Model file for the job. Use its own axes, mm. A direction names the side the tool comes from. Round coordinates to 2 decimals unless told otherwise and drop trailing zeros. Order: outer loops, then holes, each group sorted by start corner. A loop starts at its lowest first (then second) coordinate and runs counter-clockwise, first axis right, second up. Notation, with made-up numbers: (1, -3) - (46, -3) arc R23 cw to (46, 25) - close; hole circle Ø10 at (-14.75, -40). An arc over 180 degrees is marked (long way). Write item = value, one per line.
```python
from build123d import *

# Parameters (mm, degrees)
BOSS_EXTRUDE1_DEPTH   = 12.5
CHAMFER1_SIZE         = 2
HOLE1_D               = 9
CUT_EXTRUDE1_DEPTH    = 15
M4_TAPPED_HOLE1_D     = 3.3
SKETCH11_W            = 35
SKETCH11_H            = 25
CUT_EXTRUDE2_DEPTH    = 250.850455273
M8_TAPPED_HOLE2_D     = 6.8
M8_TAPPED_HOLE2_DEPTH = 19.75
M8_TAPPED_HOLE2_TIP   = 2.042926105


with BuildPart() as part:
    # Sketch1 → Boss-Extrude1 (new, symmetric)
    with BuildSketch(Plane(origin=(0, 0, 0), x_dir=(1, 0, 0), z_dir=(0, 1, 0))):
        Polygon((-75, 0), (75, 0), (75, 12), (40, 12), (40, 250), (-40, 250), (-40, 12), (-75, 12), align=None)
    extrude(amount=BOSS_EXTRUDE1_DEPTH, both=True)

    # Chamfer1
    chamfer1_edges = [part.edges().sort_by_distance(p)[0] for p in [
        (-75, 0, -12),
        (-40, 0, -250),
        (40, 0, -250),
        (75, 0, -12),
    ]]
    chamfer(chamfer1_edges, length=CHAMFER1_SIZE)

    # Hole1 (through all)
    with Locations(Plane.XY):
        with Locations((-60, 0), (60, 0)):
            Hole(HOLE1_D / 2)

    # Sketch4 → Cut-Extrude1 (cut)
    with BuildSketch(Plane(origin=(0, -12.5, 0), x_dir=(-1, 0, 0), z_dir=(0, -1, 0))):
        with BuildLine():
            Line((-13.5, 80), (-13.5, 250))
            ThreePointArc((-13.5, 250), (0, 263.5), (13.5, 250))
            Line((13.5, 250), (13.5, 80))
            ThreePointArc((13.5, 80), (0, 66.5), (-13.5, 80))
        make_face()
    extrude(amount=-CUT_EXTRUDE1_DEPTH, mode=Mode.SUBTRACT)

    # M4 Tapped Hole1 (through all)
    with Locations(Plane(origin=(0, 12.5, 0), x_dir=(1, 0, 0), z_dir=(0, 1, 0))):
        with Locations((-10, 235), (-10, 221), (10, 221), (10, 235)):
            Hole(M4_TAPPED_HOLE1_D / 2)

    # Sketch11 → Cut-Extrude2 (cut, through all)
    with BuildSketch(Plane(origin=(0, 0, -12), x_dir=(-1, 0, 0), z_dir=(0, 0, -1))):
        with Locations((-57.5, 0)):
            Rectangle(SKETCH11_W, SKETCH11_H)
        with Locations((57.5, 0)):
            Rectangle(SKETCH11_W, SKETCH11_H)
    extrude(amount=-CUT_EXTRUDE2_DEPTH, mode=Mode.SUBTRACT)

    # M8 Tapped Hole2
    with Locations(Plane.XY):
        with Locations((-25, 0), (25, 0)):
            Hole(M8_TAPPED_HOLE2_D / 2, depth=M8_TAPPED_HOLE2_DEPTH)
            with Locations((0, 0, -(M8_TAPPED_HOLE2_DEPTH + M8_TAPPED_HOLE2_TIP / 2))):  # 118° drill point
                Cone(0, M8_TAPPED_HOLE2_D / 2, M8_TAPPED_HOLE2_TIP, mode=Mode.SUBTRACT)


solid = part.part
```
1) Flat gauge pin, fed straight in: pin 1 Ø4 at (x, z) = (10, -235) entering from +Y. Where does the tip first touch, or does it go through?
Conclusion:
pin_1 = 12.5
2) Cut at B-B (y = -10.25). Write the cut outline in (x, z).
Conclusion:
outline = (-40, -248) - (-38, -250) - (-13.5, -250) - (-13.5, -80) arc R13.5 cw to (13.5, -80) - (13.5, -250) - (38, -250) - (40, -248) - (40, 0) - (-40, 0) - close
3) Wall check: line 1 along X through (y, z) = (0, -6.25); line 2 along X through (y, z) = (6.5, -235); line 3 along Z through (x, y) = (-10, 10). Give the ranges that are in metal, low to high.
Conclusion:
line_1 = -40 to -28.4, -21.6 to 21.6, 28.4 to 40
line_2 = -40 to -11.65, -8.35 to 8.35, 11.65 to 40
line_3 = -250 to -236.65, -233.35 to -222.65, -219.35 to 0
4) Mould opens along X. For faces 1 (the face through (1, 3, -250)), 2 (the face through (13.5, -5, -164)), 3 (the face through (40, 0, -122)), 4 (the face through (24.565, 0.399, -21.438)) say: +X half, -X half, draft (parallel to the pull), parting line (faces both ways), or undercut.
Conclusion:
face_1 = draft
face_2 = undercut
face_3 = +X half
face_4 = undercut
5) 3-axis set-ups, long thin cutter, end or side, ignore diameter. For faces 5 (the face through (0, 2.5, -160)), 6 (the face through (-1, 12.5, -127)), 7 (the face through (21.86, -1.3, -10.01)): which of +Z, -Z, +X, -X, +Y, -Y reach the whole face in a straight line?
Conclusion:
face_5 = -Z, -Y
face_6 = +Z, -Z, +X, -X, +Y
face_7 = +Z
6) Cut at A-A (z = -108). Write the cut outline in (x, y).
Conclusion:
outline = (-40, -12.5) - (-13.5, -12.5) - (-13.5, 2.5) - (13.5, 2.5) - (13.5, -12.5) - (40, -12.5) - (40, 12.5) - (-40, 12.5) - close
